Check sheet for the modelled part. Datum: model origin and axes. Units: mm. Round coordinates to 2 decimals unless told otherwise and drop trailing zeros. Write each loop counter-clockwise with the first axis right and the second up, starting at its lowest first coordinate (ties: lowest second). Pieces come first, ordered by that corner, then holes.
from build123d import *

# Parameters (mm, degrees)
EXTRUDE_1_DEPTH = 2


with BuildPart() as part:
    # 草图1 → 凸台-拉伸1 (new body)
    with BuildSketch(Plane.XY):
        Polygon((0, 0), (30.5, 0), (30.5, -17), (10, -40), (0, -40), align=None)
    extrude(amount=EXTRUDE_1_DEPTH)


solid = part.part
1. Sectioned sample at A-A, the plane z = 0.4. Enter the section's corners in (x, y), plus the area to 3 significant figures.
2. Scan lines: line 1 along X through (y, z) = (-30, 1.65); line 2 along Y through (x, z) = (28, 1.45); line 3 along Y through (x, z) = (23, 0.35). Record each from-to range of solid material in increasing order.
3. Sectioned sample at B-B, the plane y = -36.5. Enter the section's corners in (x, z).
4. Sectioned sample at C-C, the plane x = 28. Enter the section's corners in (y, z), plus the area to 3 significant figures.
Computed values:
1. outline: (0, -40) - (10, -40) - (30.5, -17) - (30.5, 0) - (0, 0) - close
1. area: 984 mm2
2. line 1: x = 0 to 18.91
2. line 2: y = -19.8 to 0
2. line 3: y = -25.41 to 0
3. outline: (0, 0) - (13.12, 0) - (13.12, 2) - (0, 2) - close
4. outline: (-19.8, 0) - (0, 0) - (0, 2) - (-19.8, 2) - close
4. area: 39.6 mm2
